Design review of the part built by this model. Coordinates are the model's own, in mm. A direction names the side the tool comes from. Round coordinates to 2 decimals unless told otherwise and drop trailing zeros. Write each loop counter-clockwise with the first axis right and the second up, starting at its lowest first coordinate (ties: lowest second). Pieces come first, ordered by that corner, then holes. Notation, with made-up numbers: (13, -12.75) - (48, -12.75) arc R17 cw to (48, -6.75) - close; hole circle Ø11 at (20.25, 40.25). An arc over 180 degrees is marked (long way). Use one line per item in the form item = value.
```python
from build123d import *

# Parameters (mm, degrees)
SKETCH1_W           = 42
SKETCH1_H           = 42
BOSS_EXTRUDE1_DEPTH = 15
CHAMFER1_SIZE       = 8
BOSS_EXTRUDE2_DEPTH = 9
SKETCH4_R           = 11.5
BOSS_EXTRUDE3_DEPTH = 2
SKETCH5_R           = 2.5
BOSS_EXTRUDE4_DEPTH = 22
CUT_EXTRUDE1_START  = -2
SKETCH6_R           = 4
SKETCH6_R_2         = 2.5
CUT_EXTRUDE1_DEPTH  = 2
CHAMFER2_SIZE       = 0.5
SKETCH7_R           = 2
CUT_EXTRUDE2_DEPTH  = 57.444663167


with BuildPart() as part:
    # Sketch1 → Boss-Extrude1 (new, symmetric)
    with BuildSketch(Plane.XY):
        Rectangle(SKETCH1_W, SKETCH1_H)
    extrude(amount=BOSS_EXTRUDE1_DEPTH, both=True)

    # Chamfer1
    chamfer1_edges = [part.edges().sort_by_distance(p)[0] for p in [
        (-21, 21, 0),
        (21, 21, 0),
        (21, -21, 0),
        (-21, -21, 0),
    ]]
    chamfer(chamfer1_edges, length=CHAMFER1_SIZE)

    # Sketch3 → Boss-Extrude2 (add)
    with BuildSketch(Plane.XY.offset(15)):
        Polygon((16, -21), (-16, -21), (-21, -16), (-21, 16), (-16, 21), (16, 21), (21, 16), (21, -16), align=None)
    boss_extrude2 = extrude(amount=BOSS_EXTRUDE2_DEPTH)

    # Mirror1: Boss-Extrude2 across plane
    add(boss_extrude2.mirror(Plane.XY))

    # Sketch4 → Boss-Extrude3 (add)
    with BuildSketch(Plane.XY.offset(24)):
        with Locations(Location((0, 0, 0), (0, 0, 180))):
            Circle(SKETCH4_R)
    extrude(amount=BOSS_EXTRUDE3_DEPTH)

    # Sketch5 → Boss-Extrude4 (add)
    with BuildSketch(Plane.XY.offset(26)):
        Circle(SKETCH5_R)
    extrude(amount=BOSS_EXTRUDE4_DEPTH)

    # Sketch6 → Cut-Extrude1 (cut)
    with BuildSketch(Plane.XY.offset(26).offset(CUT_EXTRUDE1_START)):
        Circle(SKETCH6_R)
        Circle(SKETCH6_R_2, mode=Mode.SUBTRACT)
    extrude(amount=CUT_EXTRUDE1_DEPTH, mode=Mode.SUBTRACT)

    # Chamfer2
    chamfer2_edges = [part.edges().sort_by_distance(p)[0] for p in [
        (-2.5, 0, 48),
    ]]
    chamfer(chamfer2_edges, length=CHAMFER2_SIZE)

    # Sketch7 → Cut-Extrude2 (cut, through all)
    with BuildSketch(Plane.XY.offset(24)):
        with Locations((15.5, 15.5)):
            Circle(SKETCH7_R)
        with Locations((15.5, -15.5)):
            Circle(SKETCH7_R)
        with Locations((-15.5, -15.5)):
            Circle(SKETCH7_R)
        with Locations((-15.5, 15.5)):
            Circle(SKETCH7_R)
    extrude(amount=-CUT_EXTRUDE2_DEPTH, mode=Mode.SUBTRACT)


solid = part.part
```
Q1. To check wall thickness, follow line 1 along Y through (x, z) = (0, 25); line 2 along X through (y, z) = (15, -9); line 3 along Y through (x, z) = (-15.5, 2). State the ranges of each line that lie inside material, in increasing order. Write a range as from..to.
Calculated:
line_1 = -11.5..-4, -2.5..2.5, 4..11.5
line_2 = -19..-17.44, -13.56..13.56, 17.44..19
line_3 = -18.5..-17.5, -13.5..13.5, 17.5..18.5
Q2. For P1, Ø4, axis at x = -6, y = -0.5, coming from the +Z side; P2, Ø9, axis at x = 16, y = 16, coming from the +Z side; P3, Ø2.5, axis at x = 15.5, y = 15, coming from the -Z side; P4, Ø1.5, axis at x = -14.5, z = 4, coming from the +Y side, all flat-tipped, find the tip position at first contact; note any pin that passes through.
Calculated:
P1 = 26
P2 = 24
P3 = through
P4 = 20.25
Q3. Machinability: for faces 4 (the flat face through (18, 16, 0)), 5 (the flat face through (-18, 18, 15)), 6 (the flat face through (-9, -9, 24)), which of the approach directions +Z, -Z, +X, -X, +Y, -Y give a long, thin tool a straight path to every point of the face, cutting with its end or side? Answer none if there is none.
Calculated:
face_4 = +X, +Y
face_5 = -X, +Y
face_6 = +Z
Q4. We need section D-D on y = -9.5. Write out the cut boundary in (x, z).
Calculated:
outline = (-21, -24) - (21, -24) - (21, 24) - (6.48, 24) - (6.48, 26) - (-6.48, 26) - (-6.48, 24) - (-21, 24) - close
Q5. We need section C-C on x = -10. Write out the cut boundary in (y, z).
Calculated:
outline = (-21, -24) - (21, -24) - (21, 24) - (5.68, 24) - (5.68, 26) - (-5.68, 26) - (-5.68, 24) - (-21, 24) - close
Q6. We need section B-B on z = 3.5. Write out the cut boundary in (x, y), then the cut area to 3 significant figures.
Calculated:
outline = (-21, -13) - (-13, -21) - (13, -21) - (21, -13) - (21, 13) - (13, 21) - (-13, 21) - (-21, 13) - close; hole circle Ø4 at (-15.5, -15.5); hole circle Ø4 at (-15.5, 15.5); hole circle Ø4 at (15.5, -15.5); hole circle Ø4 at (15.5, 15.5)
area = 1,590 mm2
Q7. Draft analysis for pull direction Z (two halves, no side actions). For faces 1 (the flat face through (-18, -18, -15)), 2 (the flat face through (2, 2, 24)), 3 (the cylindrical face through (-15.76, 17.483, 0.336)), state which applies: released by +Z, released by -Z, zero draft, split by the parting line, or undercut.
Calculated:
face_1 = undercut
face_2 = released by +Z
face_3 = zero draft
Q8. We need section A-A on y = 0. Write out the cut boundary in (x, z), then the cut area to 3 significant figures.
Calculated:
outline = (-21, -24) - (21, -24) - (21, 24) - (11.5, 24) - (11.5, 26) - (4, 26) - (4, 24) - (2.5, 24) - (2.5, 47.5) - (2, 48) - (-2, 48) - (-2.5, 47.5) - (-2.5, 24) - (-4, 24) - (-4, 26) - (-11.5, 26) - (-11.5, 24) - (-21, 24) - close
area = 2,170 mm2
